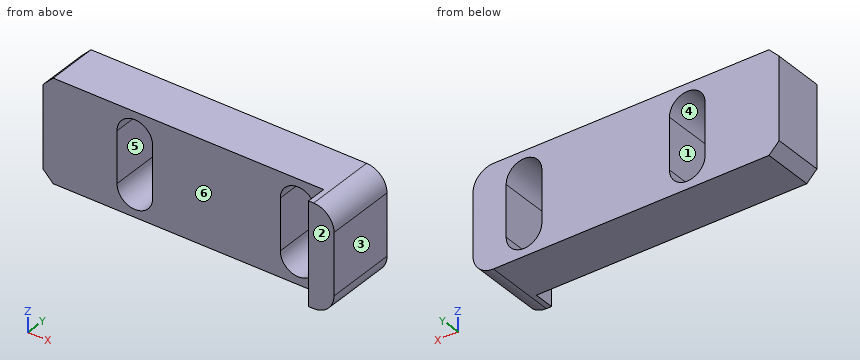
from build123d import *

# Parameters (mm, degrees)
BOSS_EXTRUDE1_DEPTH = 5
CUT_EXTRUDE1_DEPTH  = 31.822070015
FILLET1_R           = 2
CHAMFER1_SIZE       = 1


with BuildPart() as part:
    # Sketch1 → Boss-Extrude1 (new, symmetric)
    with BuildSketch(Plane.XY):
        Polygon((0, 0), (-30, 0), (-30, -5), (-2.5, -5), (-2.5, -7), (0, -7), align=None)
    extrude(amount=BOSS_EXTRUDE1_DEPTH, both=True)

    # Sketch2 → Cut-Extrude1 (cut, through all)
    with BuildSketch(Plane.XZ.offset(5)):
        with BuildLine():
            Line((-19.25, 2.5), (-19.25, -2.5))
            ThreePointArc((-19.25, -2.5), (-21, -4.25), (-22.75, -2.5))
            Line((-22.75, -2.5), (-22.75, 2.5))
            ThreePointArc((-22.75, 2.5), (-21, 4.25), (-19.25, 2.5))
        make_face()
        with BuildLine():
            Line((-3.25, 2.5), (-3.25, -2.5))
            ThreePointArc((-3.25, -2.5), (-5, -4.25), (-6.75, -2.5))
            Line((-6.75, -2.5), (-6.75, 2.5))
            ThreePointArc((-6.75, 2.5), (-5, 4.25), (-3.25, 2.5))
        make_face()
    extrude(amount=-CUT_EXTRUDE1_DEPTH, mode=Mode.SUBTRACT)

    # Fillet1
    fillet1_edges = [part.edges().sort_by_distance(p)[0] for p in [
        (0, -3.5, 5),
        (0, -3.5, -5),
    ]]
    fillet(fillet1_edges, radius=FILLET1_R)

    # Chamfer1
    chamfer1_edges = [part.edges().sort_by_distance(p)[0] for p in [
        (-30, -2.5, 5),
        (-30, -2.5, -5),
    ]]
    chamfer(chamfer1_edges, length=CHAMFER1_SIZE)


solid = part.part
Read the model definition and answer for the solid it produces. Units are mm, in the model's axes. Face numbers are marked on the shaded views. A direction names the side the tool comes from. Round coordinates to 2 decimals unless told otherwise and drop trailing zeros. Loops run counter-clockwise (first coordinate to the right, second up) from the corner with the lowest first, then second, coordinate; pieces in that order, holes last.
Q1. Which of the six approach directions +Z, -Z, +X, -X, +Y, -Y give full straight-line access (tool end or side, diameter ignored) to the marked faces 1 and 2?
Q2. Each of these flat-tipped pins is pushed along its axis until it touches: pin 1 (3 mm diameter, centred on x = -19.5, z = 2.5, fed in from -Y); pin 2 (2 mm diameter, centred on y = -6.5, z = 2, fed in from -X). Where does it stop, or does it pass through?
Q3. Consider probe 1 along X at (y, z) = (-4, -0.75); probe 2 along Y at (x, z) = (-15.25, -4.25). Determine where each line is inside the solid, lowest interval first.
Q4. Section B-B on y = -1.5 is taken. Write down the section's boundary in (x, z).
Q5. Section D-D on y = -5.75 is taken. Write down the section's boundary in (x, z).
Q6. Section C-C on z = 1.5 is taken. Write down the section's boundary in (x, y).
Q7. Section A-A on x = -21 is taken. Write down the section's boundary in (y, z), and give its area (3 significant figures).
Q8. Determine the mould class of the marked faces 3, 4, 5 and 6 for opening direction X: released by +X, released by -X, zero draft, split by the parting line, or undercut.
Output:
1. face 1: +Y, -Y
1. face 2: +Z, -Z, +X, -X, -Y
2. pin 1: stops at y = -5
2. pin 2: stops at x = -2.5
3. probe 1: x = -30 to -22.75, -19.25 to -6.75, -3.25 to 0
3. probe 2: y = -5 to 0
4. outline: (-30, -4) - (-29, -5) - (-2, -5) arc R2 ccw to (0, -3) - (0, 3) arc R2 ccw to (-2, 5) - (-29, 5) - (-30, 4) - close; hole (-22.75, -2.5) arc R1.75 ccw to (-19.25, -2.5) - (-19.25, 2.5) arc R1.75 ccw to (-22.75, 2.5) - close; hole (-6.75, -2.5) arc R1.75 ccw to (-3.25, -2.5) - (-3.25, 2.5) arc R1.75 ccw to (-6.75, 2.5) - close
5. outline: (-2.5, -5) - (-2, -5) arc R2 ccw to (0, -3) - (0, 3) arc R2 ccw to (-2, 5) - (-2.5, 5) - close
6. outline: (-30, -5) - (-22.75, -5) - (-22.75, 0) - (-30, 0) - close; (-19.25, -5) - (-6.75, -5) - (-6.75, 0) - (-19.25, 0) - close; (-3.25, -5) - (-2.5, -5) - (-2.5, -7) - (0, -7) - (0, 0) - (-3.25, 0) - close
7. outline: (-5, -5) - (0, -5) - (0, -4.25) - (-5, -4.25) - close; (-5, 4.25) - (0, 4.25) - (0, 5) - (-5, 5) - close
7. area: 7.50 mm2
8. face 3: released by +X
8. face 4: undercut
8. face 5: undercut
8. face 6: zero draft
